Check sheet for the modelled part. Datum: model origin and axes. Units: mm. Face numbers are marked on the shaded views. A direction names the side the tool comes from. Coordinates: 2 decimals unless noted, no trailing zeros. Loops run counter-clockwise (first coordinate to the right, second up) from the corner with the lowest first, then second, coordinate; pieces in that order, holes last. Notation, with made-up numbers: (34.25, 89.5) -> (83.25, 89.5) arc R21 cw to (83.25, 126.5) -> close; hole circle Ø10 at (-0.75, 5.25). An arc over 180 degrees is marked (long way). Use CSV: the item, a comma, the result in double quotes.
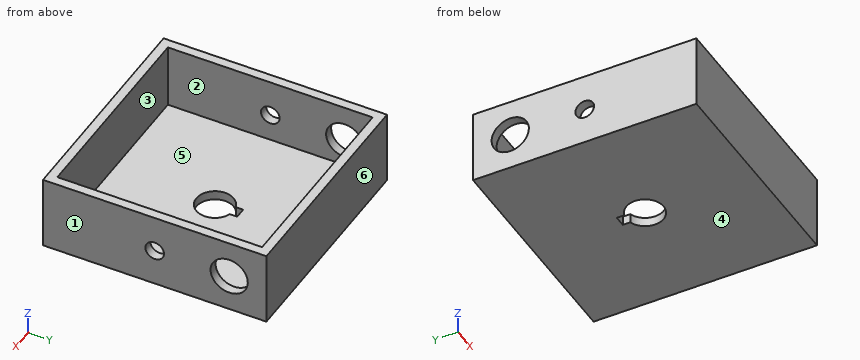
```python
from build123d import *

# Parameters (mm, degrees)
SKETCH_1_W          = 120
SKETCH_1_H          = 120
EXTRUDE_1_DEPTH     = 40
SKETCH_3_R          = 10
SKETCH_3_R_2        = 5
CUT_EXTRUDE_1_DEPTH = 141
SKETCH_4_W          = 110
SKETCH_4_H          = 110
CUT_EXTRUDE_3_DEPTH = 35
CUT_EXTRUDE_4_DEPTH = 94.808315196


with BuildPart() as part:
    # 草图1 → 凸台-拉伸1 (new body)
    with BuildSketch(Plane.XY):
        Rectangle(SKETCH_1_W, SKETCH_1_H)
    extrude(amount=EXTRUDE_1_DEPTH)

    # 草图3 → 切除-拉伸1 (cut, through all)
    with BuildSketch(Plane(origin=(60, 0, 0), x_dir=(0, 0, -1), z_dir=(1, 0, 0))):
        with Locations((-20, 40)):
            Circle(SKETCH_3_R)
        with Locations((-20, 0)):
            Circle(SKETCH_3_R_2)
    extrude(amount=-CUT_EXTRUDE_1_DEPTH, mode=Mode.SUBTRACT)

    # 草图4 → 切除-拉伸3 (cut)
    with BuildSketch(Plane.XY.offset(40)):
        Rectangle(SKETCH_4_W, SKETCH_4_H)
    extrude(amount=-CUT_EXTRUDE_3_DEPTH, mode=Mode.SUBTRACT)

    # 草图5 → 切除-拉伸4 (cut, through all)
    with BuildSketch(Plane(origin=(0, 0, 0), x_dir=(-1, 0, 0), z_dir=(0, 0, -1))):
        with BuildLine():
            Line((-3, 9.539392014), (-3, 13.539392014))
            Line((-3, 13.539392014), (3, 13.539392014))
            Line((3, 13.539392014), (3, 9.539392014))
            ThreePointArc((3, 9.539392014), (0, -10), (-3, 9.539392014))
        make_face()
    extrude(amount=-CUT_EXTRUDE_4_DEPTH, mode=Mode.SUBTRACT)


solid = part.part
```
1) Cross-section at A-A on z = 20. Record the boundary of the cut face in (x, y).
Answer below:
outline,"(-60, -60) -> (60, -60) -> (60, -5) -> (55, -5) -> (55, -55) -> (-55, -55) -> (-55, -5) -> (-60, -5) -> close; (-60, 5) -> (-55, 5) -> (-55, 30) -> (-60, 30) -> close; (-60, 50) -> (-55, 50) -> (-55, 55) -> (55, 55) -> (55, 50) -> (60, 50) -> (60, 60) -> (-60, 60) -> close; (55, 5) -> (60, 5) -> (60, 30) -> (55, 30) -> close"
2) Cross-section at C-C on x = 0. Record the boundary of the cut face in (y, z).
Answer below:
outline,"(-60, 0) -> (-10, 0) -> (-10, 5) -> (-55, 5) -> (-55, 40) -> (-60, 40) -> close; (13.54, 0) -> (60, 0) -> (60, 40) -> (55, 40) -> (55, 5) -> (13.54, 5) -> close"
3) Cross-section at D-D on y = 0. Record the boundary of the cut face in (x, z), and give its area (3 significant figures).
Answer below:
outline,"(-60, 0) -> (-10, 0) -> (-10, 5) -> (-55, 5) -> (-55, 15) -> (-60, 15) -> close; (-60, 25) -> (-55, 25) -> (-55, 40) -> (-60, 40) -> close; (10, 0) -> (60, 0) -> (60, 15) -> (55, 15) -> (55, 5) -> (10, 5) -> close; (55, 25) -> (60, 25) -> (60, 40) -> (55, 40) -> close"
area,"750 mm²"
4) Access from +Z, -Z, +X, -X, +Y, -Y to the whole of each face (thin tool, end or side, straight path). Record for the marked faces 5 and 6.
Answer below:
face 5,"+Z"
face 6,"+Z, -Z, +X, -X, +Y"
5) Draft check along X on the marked faces 1, 2, 3 and 4. Enter one of: released by +X, released by -X, zero draft, split by the parting line, or undercut.
Answer below:
face 1,"released by +X"
face 2,"undercut"
face 3,"undercut"
face 4,"zero draft"
6) Go/stop test with flat-tipped pins: pin 1 Ø12 at (y, z) = (40, 20) entering from +X (1 decimal); pin 2 Ø1 at (x, y) = (34, -34) entering from +Z. Record where each tip stops, or that it passes through.
Answer below:
pin 1,"passes through"
pin 2,"stops at z = 5"
7) Cross-section at B-B on y = 40. Record the boundary of the cut face in (x, z), and give its area (3 significant figures).
Answer below:
outline,"(-60, 0) -> (60, 0) -> (60, 10) -> (55, 10) -> (55, 5) -> (-55, 5) -> (-55, 10) -> (-60, 10) -> close; (-60, 30) -> (-55, 30) -> (-55, 40) -> (-60, 40) -> close; (55, 30) -> (60, 30) -> (60, 40) -> (55, 40) -> close"
area,"750 mm²"
8) Thickness scan on line 1 along Y through (x, z) = (-58.35, 20); line 2 along Y through (x, z) = (-29, 10.5). Record the ranges inside material, lowest first. Write a range as from..to.
Answer below:
line 1,"y = -60..-5, 5..30, 50..60"
line 2,"y = -60..-55, 55..60"
